Work out the finished part from the listing and answer in its coordinate system (mm). Face numbers are marked on the shaded views. A direction names the side the tool comes from. Round coordinates to 2 decimals unless told otherwise and drop trailing zeros. Loops run counter-clockwise (first coordinate to the right, second up) from the corner with the lowest first, then second, coordinate; pieces in that order, holes last. Notation, with made-up numbers: (-12, 85) - (12, 85) arc R5 cw to (12, 93) - close; hole circle Ø8 at (54, 51). An arc over 180 degrees is marked (long way). Return JSON: item names as keys, results as strings.
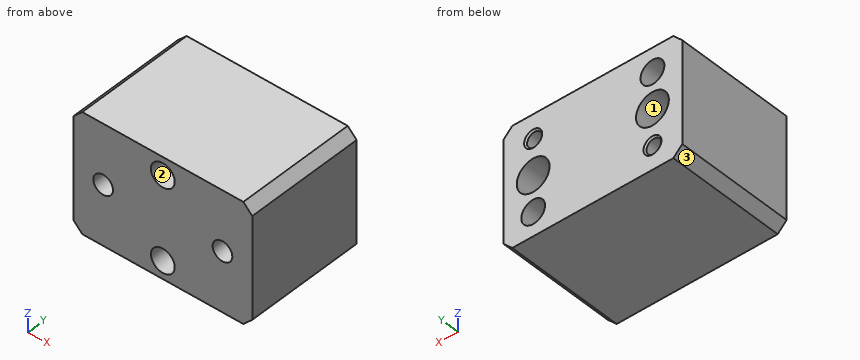
from build123d import *

# Parameters (mm, degrees)
SKETCH1_W                   = 60
SKETCH1_H                   = 40
BOSS_EXTRUDE1_DEPTH         = 40
CHAMFER1_SIZE               = 3
M6_TAPPED_HOLE1_D           = 5
M6_TAPPED_HOLE1_DEPTH       = 10.497848452
M6_TAPPED_HOLE1_CSINK_D     = 6.05
M6_TAPPED_HOLE1_CSINK_ANGLE = 90
M6_TAPPED_HOLE1_TIP         = 1.502151548
HOLE1_D                     = 6.6
HOLE1_CBORE_D               = 11
HOLE1_CBORE_DEPTH           = 27
HOLE2_D                     = 8
HOLE2_DEPTH                 = 9
HOLE3_D                     = 8
HOLE3_DEPTH                 = 8.5


with BuildPart() as part:
    # Sketch1 → Boss-Extrude1 (new body)
    with BuildSketch(Plane.XY):
        with Locations((-2.229013427, 0.789473684)):
            Rectangle(SKETCH1_W, SKETCH1_H)
    extrude(amount=BOSS_EXTRUDE1_DEPTH)

    # Chamfer1
    chamfer1_edges = [part.edges().sort_by_distance(p)[0] for p in [
        (27.770986573, 0.789473684, 40),
        (-32.229013427, 0.789473684, 40),
        (27.770986573, 0.789473684, 0),
        (-32.229013427, 0.789473684, 0),
    ]]
    chamfer(chamfer1_edges, length=CHAMFER1_SIZE)

    # M6 Tapped Hole1
    with Locations(Plane(origin=(0, 20.789473684, 0), x_dir=(1, 0, 0), z_dir=(0, 1, 0))):
        with Locations((-22.229013427, -8), (17.770986573, -32)):
            CounterSinkHole(M6_TAPPED_HOLE1_D / 2, M6_TAPPED_HOLE1_CSINK_D / 2, depth=M6_TAPPED_HOLE1_DEPTH, counter_sink_angle=M6_TAPPED_HOLE1_CSINK_ANGLE)
            with Locations((0, 0, -(M6_TAPPED_HOLE1_DEPTH + M6_TAPPED_HOLE1_TIP / 2))):  # 118° drill point
                Cone(0, M6_TAPPED_HOLE1_D / 2, M6_TAPPED_HOLE1_TIP, mode=Mode.SUBTRACT)

    # Hole1 (through all)
    with Locations(Plane(origin=(0, 20.789473684, 0), x_dir=(1, 0, 0), z_dir=(0, 1, 0))):
        with Locations((-22.229013427, -20), (17.770986573, -20)):
            CounterBoreHole(HOLE1_D / 2, HOLE1_CBORE_D / 2, HOLE1_CBORE_DEPTH)

    # Hole2
    with Locations(Plane(origin=(0, 20.789473684, 0), x_dir=(1, 0, 0), z_dir=(0, 1, 0))):
        with Locations((17.770986573, -8), (-22.229013427, -32)):
            Hole(HOLE2_D / 2, depth=HOLE2_DEPTH)

    # Hole3
    with Locations(Plane(origin=(0, -19.210526316, 0), x_dir=(-1, 0, 0), z_dir=(0, -1, 0))):
        with Locations((2.229013427, -34), (2.229013427, -6)):
            Hole(HOLE3_D / 2, depth=HOLE3_DEPTH)


solid = part.part
1) Flat-ended cylindrical pins translate along their axes: pin 1 (10.5 mm diameter, centred on x = 17.77, z = 20, fed in from +Y); pin 2 (2.5 mm diameter, centred on x = -20.5, z = 34, fed in from +Y); pin 3 (7 mm diameter, centred on x = -2.23, z = 34, fed in from -Y). Find the tip coordinate at first contact, or state that the pin passes through.
Verdict:
{"pin 1": "stops at y = -6.21", "pin 2": "stops at y = 11.79", "pin 3": "stops at y = -10.71"}
2) Section D-D (y = -9) is taken. Give the vertices of the cut face in (x, z).
Verdict:
{"outline": "(-32.23, 3) - (-29.23, 0) - (24.77, 0) - (27.77, 3) - (27.77, 37) - (24.77, 40) - (-29.23, 40) - (-32.23, 37) - close; hole circle Ø6.6 at (-22.23, 20); hole circle Ø6.6 at (17.77, 20)"}
3) Section C-C (y = 6.5) is taken. Give the vertices of the cut face in (x, z).
Verdict:
{"outline": "(-32.23, 3) - (-29.23, 0) - (24.77, 0) - (27.77, 3) - (27.77, 37) - (24.77, 40) - (-29.23, 40) - (-32.23, 37) - close; hole circle Ø11 at (-22.23, 20); hole circle Ø11 at (17.77, 20)"}
4) Section A-A (y = -13) is taken. Give the vertices of the cut face in (x, z), and give its area (3 significant figures).
Verdict:
{"outline": "(-32.23, 3) - (-29.23, 0) - (24.77, 0) - (27.77, 3) - (27.77, 37) - (24.77, 40) - (-29.23, 40) - (-32.23, 37) - close; hole circle Ø6.6 at (-22.23, 20); hole circle Ø8 at (-2.23, 6); hole circle Ø8 at (-2.23, 34); hole circle Ø6.6 at (17.77, 20)", "area": "2,210 mm2"}
5) Section B-B (z = 20) is taken. Give the vertices of the cut face in (x, y), and give its area (3 significant figures).
Verdict:
{"outline": "(-32.23, -19.21) - (-25.53, -19.21) - (-25.53, -6.21) - (-27.73, -6.21) - (-27.73, 20.79) - (-32.23, 20.79) - close; (-18.93, -19.21) - (14.47, -19.21) - (14.47, -6.21) - (12.27, -6.21) - (12.27, 20.79) - (-16.73, 20.79) - (-16.73, -6.21) - (-18.93, -6.21) - close; (21.07, -19.21) - (27.77, -19.21) - (27.77, 20.79) - (23.27, 20.79) - (23.27, -6.21) - (21.07, -6.21) - close", "area": "1,630 mm2"}
6) Find the intervals of material crossed by L1, parallel to X at y = 17.5, z = 20; L2, parallel to X at y = -13.5, z = 20; L3, parallel to Z at x = -21, y = 14, in increasing order.
Verdict:
{"L1": "x = -32.23 to -27.73, -16.73 to 12.27, 23.27 to 27.77", "L2": "x = -32.23 to -25.53, -18.93 to 14.47, 21.07 to 27.77", "L3": "z = 0 to 5.82, 10.18 to 14.64, 25.36 to 28.19, 35.81 to 40"}
7) A tool of negligible diameter and unlimited length cuts with its end or side. For the marked faces 1, 2 and 3, from which of +Z, -Z, +X, -X, +Y, -Y can it reach the whole face along a straight path? Write none if from no direction.
Verdict:
{"face 1": "+Y", "face 2": "-Y", "face 3": "-Z, -X, +Y, -Y"}
